Could you check a few things on this model? Use its own coordinates, in mm. A direction names the side the tool comes from. Round coordinates to 2 decimals unless told otherwise and drop trailing zeros. Loops run counter-clockwise (first coordinate to the right, second up) from the corner with the lowest first, then second, coordinate; pieces in that order, holes last. Notation, with made-up numbers: (3, 28.25) -> (8, 28.25) arc R19 cw to (8, 61.25) -> close; hole circle Ø6 at (-1.5, 21.5). An arc over 180 degrees is marked (long way). One line per item, written item: value.
```python
from build123d import *

# Parameters (mm, degrees)
EXTRUDE_1_DEPTH    = 260
HOLE_WIZARD_M5_1_D = 5.5
HOLE_WIZARD_M5_2_D = 5.5
HOLE_WIZARD_M6_1_D = 6.6
HOLE_WIZARD_M6_2_D = 6.6
HOLE_WIZARD_M4_1_D = 3.3
HOLE_WIZARD_M4_2_D = 3.3


with BuildPart() as part:
    # 草图1 → 凸台-拉伸1 (new body)
    with BuildSketch(Plane(origin=(0, 0, 0), x_dir=(1, 0, 0), z_dir=(0, 1, 0))):
        Polygon((0, 0), (50, 0), (50, 3), (3, 3), (3, 50), (0, 50), align=None)
    extrude(amount=EXTRUDE_1_DEPTH)

    # M5 间隙孔1 (through all)
    with Locations(Plane(origin=(0, 0, -3), x_dir=(-1, 0, 0), z_dir=(0, 0, -1))):
        with Locations((-30, 250), (-30, 215), (-30, 220), (-30, 185)):
            Hole(HOLE_WIZARD_M5_1_D / 2)

    # M5 间隙孔2 (through all)
    with Locations(Plane(origin=(3, 0, 0), x_dir=(0, 0, -1), z_dir=(1, 0, 0))):
        with Locations((30, 220), (30, 185), (30, 250), (30, 215)):
            Hole(HOLE_WIZARD_M5_2_D / 2)

    # M6 间隙孔1 (through all)
    with Locations(Plane.XY):
        with Locations((25, 65), (25, 25)):
            Hole(HOLE_WIZARD_M6_1_D / 2)

    # M6 间隙孔2 (through all)
    with Locations(Plane.ZY):
        with Locations((-25, 65), (-25, 25)):
            Hole(HOLE_WIZARD_M6_2_D / 2)

    # M4 螺纹孔1 (through all)
    with Locations(Plane(origin=(0, 0, -3), x_dir=(-1, 0, 0), z_dir=(0, 0, -1))):
        with Locations((-44, 250), (-44, 167.5), (-44, 85)):
            Hole(HOLE_WIZARD_M4_1_D / 2)

    # M4 螺纹孔2 (through all)
    with Locations(Plane(origin=(3, 0, 0), x_dir=(0, 0, -1), z_dir=(1, 0, 0))):
        with Locations((44, 250), (44, 167.5), (44, 85)):
            Hole(HOLE_WIZARD_M4_2_D / 2)


solid = part.part
```
Item 1: If we mould it in two halves opening along Z, with no side actions, what happens to faces 3 (the face through (1.48, 212.25, -30.1)), 4 (the face through (1.521, 67.783, -26.774)), 5 (the face through (23.48, 22.07, -1.52)), 6 (the face through (27, 128, -3))? For each: released by +Z, released by -Z, zero draft, split by the parting line, or undercut.
Output:
face 3: undercut
face 4: undercut
face 5: zero draft
face 6: released by -Z
Item 2: If we section it at C-C on y = 104: List the corners of the cut face in (x, z) for me.
Output:
outline: (0, -50) -> (3, -50) -> (3, -3) -> (50, -3) -> (50, 0) -> (0, 0) -> close
Item 3: I need wall thicknesses on line 1 (Y direction, x = 2.15, z = -30); line 2 (X direction, y = 42.5, z = -34); line 3 (Z direction, x = 19.5, y = 128). Which ranges of each line are inside material? Lowest first, please. Write a range as from..to.
Output:
line 1: y = 0..182.25, 187.75..212.25, 222.75..247.25, 252.75..260
line 2: x = 0..3
line 3: z = -3..0
Item 4: If we section it at B-B on z = -25: List the corners of the cut face in (x, y) for me, plus the area to 3 significant figures.
Output:
outline: (0, 0) -> (3, 0) -> (3, 21.7) -> (0, 21.7) -> close; (0, 28.3) -> (3, 28.3) -> (3, 61.7) -> (0, 61.7) -> close; (0, 68.3) -> (3, 68.3) -> (3, 260) -> (0, 260) -> close
area: 740 mm²
Item 5: If we section it at A-A on y = 65: List the corners of the cut face in (x, z) for me, plus the area to 3 significant figures.
Output:
outline: (0, -50) -> (3, -50) -> (3, -28.3) -> (0, -28.3) -> close; (0, -21.7) -> (3, -21.7) -> (3, -3) -> (21.7, -3) -> (21.7, 0) -> (0, 0) -> close; (28.3, -3) -> (50, -3) -> (50, 0) -> (28.3, 0) -> close
area: 251 mm²
Item 6: If we section it at D-D on x = 16: List the corners of the cut face in (y, z) for me.
Output:
outline: (0, -3) -> (260, -3) -> (260, 0) -> (0, 0) -> close
Item 7: For faces 1 (the face through (29.404, 247.315, -1.479)), 2 (the face through (3, 128, -26)), which set-ups out of +Z, -Z, +X, -X, +Y, -Y let a thin tool reach every point of the face, with its end or its side?
Output:
face 1: +Z, -Z
face 2: -Z, +X, +Y, -Y
Item 8: Will these pins go through, and if not, where does the flat tip stop? pin 1 Ø4.5 at (x, y) = (30, 215) entering from -Z; pin 2 Ø7 at (y, z) = (185, -30) entering from +X; pin 3 Ø14 at (x, y) = (15, 134) entering from -Z.
Output:
pin 1: passes through
pin 2: stops at x = 3
pin 3: stops at z = -3
